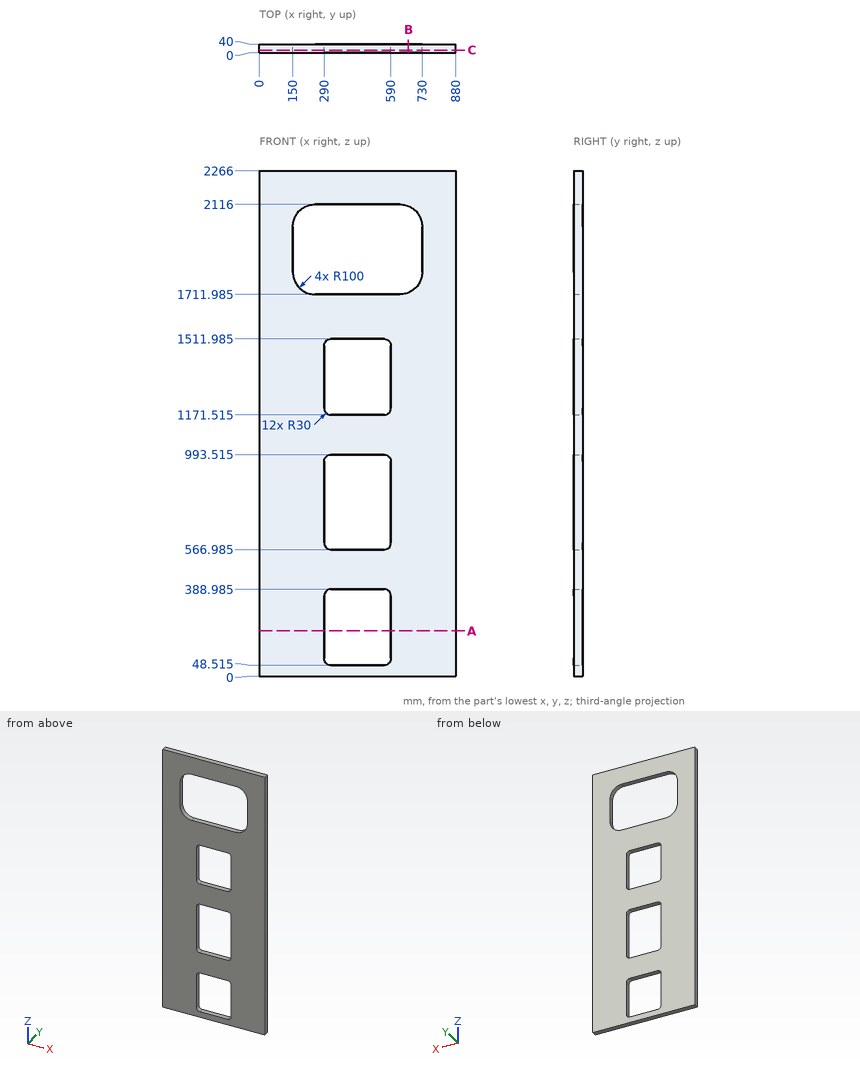
The drawing under review shows one solid part. Ordinate dimensions are in mm from its lowest x, y, z. Round coordinates to 2 decimals unless told otherwise and drop trailing zeros. Write each loop counter-clockwise with the first axis right and the second up, starting at its lowest first coordinate (ties: lowest second). Pieces come first, ordered by that corner, then holes.
(1) We need section C-C on y = 12. Give the number of separate pieces and of enclosed holes in the cut face, and give its area (3 significant figures).
(2) We need section B-B on x = 668.5. Give the boundary of the cut face in (y, z).
(3) Wall thickness on L1, parallel to Z at x = 497, y = 12 (1 decimal); L2, parallel to X at y = 20, z = 1208.5; L3, parallel to X at y = 23.5, z = 1919.5: over which ranges is each line inside the solid? List them lowest first.
(4) We need section A-A on z = 202. Give the boundary of the cut face in (x, y), and give its area (3 significant figures).
Findings below:
1. separate pieces: 1
1. enclosed holes: 4
1. area: 1,440,000 mm2
2. outline: (0, 0) - (40, 0) - (40, 1719.69) - (0, 1719.69) - close; (0, 2108.29) - (40, 2108.29) - (40, 2266) - (0, 2266) - close
3. L1: z = 0 to 48.5, 389 to 567, 993.5 to 1171.5, 1512 to 1712, 2116 to 2266
3. L2: x = 0 to 290, 590 to 880
3. L3: x = 0 to 150, 730 to 880
4. outline: (0, 0) - (290, 0) - (290, 40) - (0, 40) - close; (590, 0) - (880, 0) - (880, 40) - (590, 40) - close
4. area: 23,200 mm2
